CAD build for the part. Positions are in the model's coordinates, mm. Coordinates: 2 decimals unless noted, no trailing zeros. Order: outer loops, then holes, each group sorted by start corner. A loop starts at its lowest first (then second) coordinate and runs counter-clockwise, first axis right, second up. Notation, with made-up numbers: M 84.25,34.25 L 92.25,34.25 A11 ccw 92.25,42.25 Z; hole C 78.5,-30 d2. An arc over 180 degrees is marked long. Write item = value, one per line. Start each with the question number.
```python
from build123d import *

# Parameters (mm, degrees)
BOSS_EXTRUDE1_DEPTH     = 2270
CUT_EXTRUDE1_DEPTH      = 2271.600140932
CUT_EXTRUDE1_DEPTH_BACK = 2271.600140932


with BuildPart() as part:
    # Sketch1 → Boss-Extrude1 (new body)
    with BuildSketch(Plane(origin=(0, 0, 0), x_dir=(1, 0, 0), z_dir=(0, 1, 0))):
        with BuildLine():
            Line((-21.55, -15), (21.55, -15))
            ThreePointArc((21.55, -15), (23.989518395, -13.989518395), (25, -11.55))
            Line((25, -11.55), (25, 11.55))
            ThreePointArc((25, 11.55), (23.989518395, 13.989518395), (21.55, 15))
            Line((21.55, 15), (-21.55, 15))
            ThreePointArc((-21.55, 15), (-23.989518395, 13.989518395), (-25, 11.55))
            Line((-25, 11.55), (-25, -11.55))
            ThreePointArc((-25, -11.55), (-23.989518395, -13.989518395), (-21.55, -15))
        make_face()
        with BuildLine():
            Line((-21.55, -12.7), (21.55, -12.7))
            ThreePointArc((21.55, -12.7), (22.363172798, -12.363172798), (22.7, -11.55))
            Line((22.7, -11.55), (22.7, 11.55))
            ThreePointArc((22.7, 11.55), (22.363172798, 12.363172798), (21.55, 12.7))
            Line((21.55, 12.7), (-21.55, 12.7))
            ThreePointArc((-21.55, 12.7), (-22.363172798, 12.363172798), (-22.7, 11.55))
            Line((-22.7, 11.55), (-22.7, -11.55))
            ThreePointArc((-22.7, -11.55), (-22.363172798, -12.363172798), (-21.55, -12.7))
        make_face(mode=Mode.SUBTRACT)
    extrude(amount=BOSS_EXTRUDE1_DEPTH)

    # Sketch2 → Cut-Extrude1 (cut, two sides: drawn at the far end of the back side and taken through both)
    with BuildSketch(Plane(origin=(25, 0, 0), x_dir=(0, 0, -1), z_dir=(1, 0, 0)).offset(-CUT_EXTRUDE1_DEPTH_BACK)):
        Polygon((15, 2270), (-15, 2240), (-15, 2270), align=None)
        Polygon((15, 0), (-15, 0), (-15, 30), align=None)
    extrude(amount=CUT_EXTRUDE1_DEPTH + CUT_EXTRUDE1_DEPTH_BACK, mode=Mode.SUBTRACT)


solid = part.part
```
1. Slice it at A-A (z = 0.25). Write the cut outline in (x, y), plus the area to 3 significant figures.
2. Mould opens along Z. For faces 1 (the flat face through (0, 1119, -15)), 2 (the flat face through (0, 1120, 15)), 3 (the flat face through (0, 1119, -12.7)) say: released by +Z, released by -Z, zero draft, split by the parting line, or undercut.
3. Slice it at B-B (x = -12.5). Write the cut outline in (y, z).
4. Flat gauge pin, fed straight in: pin 1 (8 mm diameter, centred on x = 2.5, z = -7.5, fed in from +Y). Where does the tip first touch, or does it go through?
5. Probe L1, parallel to Z at x = -5, y = 120.5; L2, parallel to X at y = 152, z = -0.75; L3, parallel to X at y = 244.5, z = 12. List the from-to ranges inside material, lowest first.
6. Slice it at C-C (y = 1942). Write the cut outline in (x, z).
Calculated:
q1.outline = M -25,15.25 L -22.7,15.25 L -22.7,2254.75 L -25,2254.75 Z; M 22.7,15.25 L 25,15.25 L 25,2254.75 L 22.7,2254.75 Z
q1.area = 10,300 mm²
q2.face_1 = released by -Z
q2.face_2 = released by +Z
q2.face_3 = undercut
q3.outline = M 0,-15 L 2270,-15 L 2267.7,-12.7 L 2.3,-12.7 Z; M 27.7,12.7 L 2242.3,12.7 L 2240,15 L 30,15 Z
q4.pin_1 = through
q5.L1 = -15 to -12.7, 12.7 to 15
q5.L2 = -25 to -22.7, 22.7 to 25
q5.L3 = -24.97 to -22.61, 22.61 to 24.97
q6.outline = M -25,-11.55 A3.45 ccw -21.55,-15 L 21.55,-15 A3.45 ccw 25,-11.55 L 25,11.55 A3.45 ccw 21.55,15 L -21.55,15 A3.45 ccw -25,11.55 Z; hole M -22.7,-11.55 A1.15 ccw -21.55,-12.7 L 21.55,-12.7 A1.15 ccw 22.7,-11.55 L 22.7,11.55 A1.15 ccw 21.55,12.7 L -21.55,12.7 A1.15 ccw -22.7,11.55 Z
